Work out the finished part from the listing and answer in its coordinate system (mm). A direction names the side the tool comes from. Give positions to 0.01 mm unless a question says otherwise; leave off trailing zeros. Write each loop counter-clockwise with the first axis right and the second up, starting at its lowest first coordinate (ties: lowest second). Pieces come first, ordered by that corner, then holes. Notation, with made-up numbers: (50, 73.5) -> (108, 73.5) arc R28 cw to (108, 94.5) -> close; hole circle Ø5 at (31, 41.5). An arc over 180 degrees is marked (long way). Use a Markdown table: item, result. Add a question column.
Q1. Section C-C, the plane x = 32 is taken. Give the vertices of the cut face in (y, z).
Q2. For faces 1 (the face through (53, 0, -10)), 2 (the face through (58, 7.4, -4.5)), 3 (the face through (47, 4, -9)), 4 (the face through (-40.56, -8.428, 1.107)), 5 (the face through (29, 0, 6.5)), determine the directions among +Z, -Z, +X, -X, +Y, -Y from which every point of the face is accessible in a straight line to the end or side of a thin tool.
Q3. Each of these flat-tipped pins is pushed along its axis until it touches: pin 1 Ø6 at (x, y) = (5, 7.5) entering from +Z; pin 2 Ø2 at (x, y) = (-31.5, 1) entering from -Z; pin 3 Ø5 at (x, y) = (19.5, 0) entering from +Z. Where does it stop, or does it pass through?
Q4. Section D-D, the plane y = 6.25 is taken. Give the vertices of the cut face in (x, z), plus the area to 3 significant figures.
Q5. Section B-B, the plane z = 0 is taken. Give the vertices of the cut face in (x, y), plus the area to 3 significant figures.
Q6. Consider line 1 (X direction, y = 9.25, z = 0.25); line 2 (Y direction, x = -62, z = -0.25); line 3 (Y direction, x = -55.5, z = 5.75). Determine where each line is inside the solid, lowest interval first.
Q7. For a pull along X with two mould halves and no side action, classify faces 6 (the face through (70, 0, 0)), 7 (the face through (48.3, 4, -9)), 8 (the face through (63.916, 7.167, -4.57)) as pulls with the +X half, pulls with the -X half, needs draft (parallel to the pull), parting line crosses it, or undercut.
from build123d import *

# Parameters (mm, degrees)
SKETCH_1_R          = 10
EXTRUDE_1_DEPTH     = 58
SKETCH_2_R          = 8.5
EXTRUDE_2_DEPTH     = 12
EXTRUDE_START       = 80
SKETCH_3_R          = 8.5
EXTRUDE_3_DEPTH     = 80
CUT_EXTRUDE_1_DEPTH = 83.29368141
SKETCH_5_W          = 1.3
SKETCH_5_H          = 0.5


with BuildPart() as part:
    # 草图1 → 凸台-拉伸1 (new body)
    with BuildSketch(Plane(origin=(0, 0, 0), x_dir=(0, 0, -1), z_dir=(1, 0, 0))):
        with Locations(Location((0, 0, 0), (0, 0, 180))):
            Circle(SKETCH_1_R)
    extrude(amount=EXTRUDE_1_DEPTH)

    # 草图2 → 凸台-拉伸2 (add)
    with BuildSketch(Plane(origin=(58, 0, 0), x_dir=(0, 0, -1), z_dir=(1, 0, 0))):
        Circle(SKETCH_2_R)
    extrude(amount=EXTRUDE_2_DEPTH)

    # 草图3 → 凸台-拉伸3 (add)
    with BuildSketch(Plane.ZY.offset(EXTRUDE_START)):
        with Locations(Location((0, 0, 0), (0, 0, 180))):
            Circle(SKETCH_3_R)
    extrude(amount=-EXTRUDE_3_DEPTH)

    # 草图4 → 切除-拉伸1 (cut, through all)
    with BuildSketch(Plane.XY.offset(6.5)):
        with BuildLine():
            Line((13.5, 3), (43.5, 3))
            ThreePointArc((43.5, 3), (46.5, 0), (43.5, -3))
            Line((43.5, -3), (13.5, -3))
            ThreePointArc((13.5, -3), (10.5, 0), (13.5, 3))
        make_face()
    extrude(amount=CUT_EXTRUDE_1_DEPTH, mode=Mode.SUBTRACT)

    # 草图5 → 切除-旋转1 (revolve, cut)
    with BuildSketch(Plane(origin=(0, 0, 0), x_dir=(1, 0, 0), z_dir=(0, 1, 0)), mode=Mode.PRIVATE) as cut_revolve_1_sk:
        with Locations((9.35, 9.75)):
            Rectangle(SKETCH_5_W, SKETCH_5_H)
        with Locations((47.65, 9.75)):
            Rectangle(SKETCH_5_W, SKETCH_5_H)
    revolve(cut_revolve_1_sk.sketch.rotate(Axis((0, 0, 0), (1, 0, 0)), 180), axis=Axis((0, 0, 0), (1, 0, 0)), mode=Mode.SUBTRACT)


solid = part.part
Result set:
| question | item | result |
|---|---|---|
| 1 | outline | (-3, 6.5) -> (-3, 9.54) arc R10 ccw (long way) to (3, 9.54) -> (3, 6.5) -> close |
| 2 | face 1 | +X, -X |
| 2 | face 2 | +X |
| 2 | face 3 | none |
| 2 | face 4 | -X |
| 2 | face 5 | +Z |
| 3 | pin 1 | stops at z = 8.93 |
| 3 | pin 2 | stops at z = -8.5 |
| 3 | pin 3 | stops at z = 6.5 |
| 4 | outline | (-80, -5.76) -> (0, -5.76) -> (0, -7.81) -> (8.7, -7.81) -> (8.7, -7.15) -> (10, -7.15) -> (10, -7.81) -> (47, -7.81) -> (47, -7.15) -> (48.3, -7.15) -> (48.3, -7.81) -> (58, -7.81) -> (58, -5.76) -> (70, -5.76) -> (70, 5.76) -> (58, 5.76) -> (58, 7.81) -> (48.3, 7.81) -> (48.3, 7.15) -> (47, 7.15) -> (47, 7.81) -> (10, 7.81) -> (10, 7.15) -> (8.7, 7.15) -> (8.7, 7.81) -> (0, 7.81) -> (0, 5.76) -> (-80, 5.76) -> close |
| 4 | area | 1,960 mm2 |
| 5 | outline | (-80, -8.5) -> (0, -8.5) -> (0, -10) -> (8.7, -10) -> (8.7, -9.5) -> (10, -9.5) -> (10, -10) -> (47, -10) -> (47, -9.5) -> (48.3, -9.5) -> (48.3, -10) -> (58, -10) -> (58, -8.5) -> (70, -8.5) -> (70, 8.5) -> (58, 8.5) -> (58, 10) -> (48.3, 10) -> (48.3, 9.5) -> (47, 9.5) -> (47, 10) -> (10, 10) -> (10, 9.5) -> (8.7, 9.5) -> (8.7, 10) -> (0, 10) -> (0, 8.5) -> (-80, 8.5) -> close |
| 5 | area | 2,720 mm2 |
| 6 | line 1 | x = 0 to 58 |
| 6 | line 2 | y = -8.5 to 8.5 |
| 6 | line 3 | y = -6.26 to 6.26 |
| 7 | face 6 | pulls with the +X half |
| 7 | face 7 | undercut |
| 7 | face 8 | needs draft |
